The drawing under review shows one solid part. Ordinate dimensions are in mm from its lowest x, y, z. Coordinates: 2 decimals unless noted, no trailing zeros. Order: outer loops, then holes, each group sorted by start corner. A loop starts at its lowest first (then second) coordinate and runs counter-clockwise, first axis right, second up.
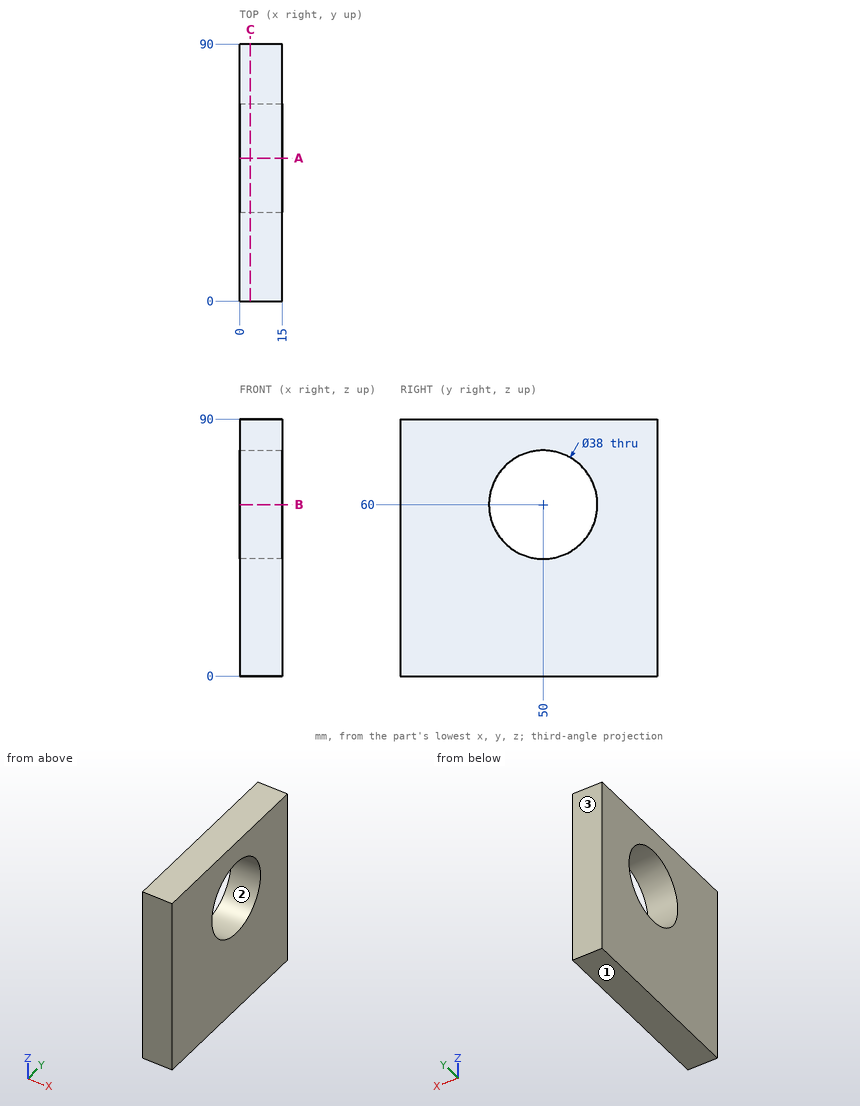
(1) Consider section A-A (y = 50). Give the boundary of the cut face in (x, z).
(2) Consider section C-C (x = 3.75). Give the boundary of the cut face in (y, z).
(3) Wall thickness on line 1 (Y direction, x = 11.25, z = 60); line 2 (Y direction, x = 4.25, z = 55); line 3 (Z direction, x = 9.5, y = 67.5): over which ranges is each line inside the solid? List them lowest first.
(4) Consider section B-B (z = 60). Give the boundary of the cut face in (x, y).
(5) The part is to be moulded in two halves that separate along Y. For the marked faces 1, 2 and 3, say which applies: +Y half, -Y half, draft (parallel to the pull), parting line (faces both ways), or undercut.
Findings:
1. outline: (0, 0) - (15, 0) - (15, 41) - (0, 41) - close; (0, 79) - (15, 79) - (15, 90) - (0, 90) - close
2. outline: (0, 0) - (90, 0) - (90, 90) - (0, 90) - close; hole circle Ø38 at (50, 60)
3. line 1: y = 0 to 31, 69 to 90
3. line 2: y = 0 to 31.67, 68.33 to 90
3. line 3: z = 0 to 52.6, 67.4 to 90
4. outline: (0, 0) - (15, 0) - (15, 31) - (0, 31) - close; (0, 69) - (15, 69) - (15, 90) - (0, 90) - close
5. face 1: draft
5. face 2: undercut
5. face 3: +Y half
